Here's how the part is built. I have some questions about the finished solid (model axes, mm). A direction names the side the tool comes from. Coordinates: 2 decimals unless noted, no trailing zeros. Loops run counter-clockwise (first coordinate to the right, second up) from the corner with the lowest first, then second, coordinate; pieces in that order, holes last. Notation, with made-up numbers: M -9,-22 L -1,-22 A12 cw -1,-4 Z; hole C 38,-26 d1. An arc over 180 degrees is marked long. Use one line per item in the form item = value. Start each with the question number.
(1) Imagine slicing it at A-A, the plane x = 0. Please give me the cut outline in (y, z).
(2) Please list where these lines run through material, in increasing order: L1, parallel to Y at x = -15, z = 2.35; L2, parallel to Z at x = 1, y = -0.75; L3, parallel to X at y = 14.25, z = 1.5.
(3) On a 3-axis mill with a long thin cutter (end or side, diameter ignored), from which of +Z, -Z, +X, -X, +Y, -Y can I reach the whole of each face in a straight line? I mean faces 5 (the flat face through (19, 0, 6)), 6 (the flat face through (-19, 0, 6)), 7 (the cylindrical face through (10.5, 0, 11.9)), 8 (the flat face through (0, 0, 18)). Say none if no direction works.
(4) Imagine slicing it at B-B, the plane z = 2.25. Please give me the cut outline in (x, y), and give its area (3 significant figures).
(5) Imagine slicing it at D-D, the plane y = 2. Please give me the cut outline in (x, z).
(6) Imagine slicing it at C-C, the plane y = 5.75. Please give me the cut outline in (x, z), and give its area (3 significant figures).
(7) Thinking about a two-plate mould opening in Z: for faces 1 (the flat face through (0, 0, 15)), 2 (the flat face through (-13.5, 0, 11.5)), 3 (the cylindrical face through (15, 0.04, 7.43)), 4 (the flat face through (0, 0, 9)), which applies, +Z half, -Z half, draft (parallel to the pull), parting line (faces both ways), or undercut?
(8) Will these pins go through, and if not, where does the flat tip stop? P1, Ø2, axis at y = 17, z = 2.5, coming from the -X side; P2, Ø5, axis at x = -12.5, y = 16, coming from the +Z side; P3, Ø0.8, axis at y = -1, z = 11.5, coming from the -X side.
```python
from build123d import *

# Parameters (mm, degrees)
BASE_PLATE_DEPTH        = 3
CLEVIS_LUGS_PROFILE_W   = 40
CLEVIS_LUGS_PROFILE_H   = 6
CLEVIS_LUGS_PROFILE_R   = 5
CLEVIS_LUGS_PROFILE_R_2 = 2.5
CLEVIS_LUGS_DEPTH       = 3


with BuildPart() as part:
    # Base Plate Profile → Base Plate (new, symmetric)
    with BuildSketch(Plane(origin=(0, 0, 0), x_dir=(1, 0, 0), z_dir=(0, 1, 0))):
        with BuildLine():
            Line((-20, 0), (20, 0))
            Line((20, 0), (20, -6))
            Line((20, -6), (18.5, -6))
            ThreePointArc((18.5, -6), (14.964466094, -7.464466094), (13.5, -11))
            Line((13.5, -11), (13.5, -12))
            ThreePointArc((13.5, -12), (11.742640687, -16.242640687), (7.5, -18))
            Line((7.5, -18), (-7.5, -18))
            ThreePointArc((-7.5, -18), (-11.742640687, -16.242640687), (-13.5, -12))
            Line((-13.5, -12), (-13.5, -11))
            ThreePointArc((-13.5, -11), (-14.964466094, -7.464466094), (-18.5, -6))
            Line((-18.5, -6), (-20, -6))
            Line((-20, -6), (-20, 0))
        make_face()
        with BuildLine():
            Line((-7.5, -9), (7.5, -9))
            ThreePointArc((7.5, -9), (10.5, -12), (7.5, -15))
            Line((7.5, -15), (-7.5, -15))
            ThreePointArc((-7.5, -15), (-10.5, -12), (-7.5, -9))
        make_face(mode=Mode.SUBTRACT)
    extrude(amount=BASE_PLATE_DEPTH, both=True)

    # Clevis Lugs Profile → Clevis Lugs (add, symmetric)
    # profile 1 of 5: a face of its own
    with BuildSketch(Plane(origin=(0, 0, 0), x_dir=(-1, 0, 0), z_dir=(0, 0, -1))):
        Rectangle(CLEVIS_LUGS_PROFILE_W, CLEVIS_LUGS_PROFILE_H)
    # profile 2 of 5: a face of its own
    with BuildSketch(Plane(origin=(0, 0, 0), x_dir=(-1, 0, 0), z_dir=(0, 0, -1))):
        with BuildLine():
            Line((-20, 15), (-20, 3))
            Line((-20, 3), (-5, 3))
            ThreePointArc((-5, 3), (-8.535533906, 4.464466094), (-10, 8))
            Line((-10, 8), (-10, 15))
            ThreePointArc((-10, 15), (-15, 10), (-20, 15))
        make_face()
    # profile 3 of 5: a face of its own
    with BuildSketch(Plane(origin=(0, 0, 0), x_dir=(-1, 0, 0), z_dir=(0, 0, -1))):
        with BuildLine():
            Line((5, 3), (20, 3))
            Line((20, 3), (20, 15))
            ThreePointArc((20, 15), (15, 10), (10, 15))
            Line((10, 15), (10, 8))
            ThreePointArc((10, 8), (8.535533906, 4.464466094), (5, 3))
        make_face()
    # profile 4 of 5: a face of its own
    with BuildSketch(Plane(origin=(0, 0, 0), x_dir=(-1, 0, 0), z_dir=(0, 0, -1))):
        with Locations((15, 15)):
            Circle(CLEVIS_LUGS_PROFILE_R)
        with Locations((15, 15)):
            Circle(CLEVIS_LUGS_PROFILE_R_2, mode=Mode.SUBTRACT)
    # profile 5 of 5: a face of its own
    with BuildSketch(Plane(origin=(0, 0, 0), x_dir=(-1, 0, 0), z_dir=(0, 0, -1))):
        with Locations((-15, 15)):
            Circle(CLEVIS_LUGS_PROFILE_R)
        with Locations((-15, 15)):
            Circle(CLEVIS_LUGS_PROFILE_R_2, mode=Mode.SUBTRACT)
    extrude(amount=CLEVIS_LUGS_DEPTH, both=True)


solid = part.part
```
Answer:
q1.outline = M -3,-3 L 3,-3 L 3,9 L -3,9 Z; M -3,15 L 3,15 L 3,18 L -3,18 Z
q2.L1 = -3 to 12.5, 17.5 to 20
q2.L2 = -3 to 9, 15 to 18
q2.L3 = -20 to -17.38, -12.62 to -10, 10 to 12.62, 17.38 to 20
q3.face_5 = +Z, +X, +Y, -Y
q3.face_6 = +Z, -X, +Y, -Y
q3.face_7 = +Y, -Y
q3.face_8 = +Z, +X, -X, +Y, -Y
q4.outline = M -20,-3 L 20,-3 L 20,15 A5 ccw 10,15 L 10,8 A5 cw 5,3 L -5,3 A5 cw -10,8 L -10,15 A5 ccw -20,15 Z; hole C -15,15 d5; hole C 15,15 d5
q4.area = 530 mm²
q5.outline = M -20,-3 L 20,-3 L 20,6 L 18.5,6 A5 cw 13.5,11 L 13.5,12 A6 ccw 7.5,18 L -7.5,18 A6 ccw -13.5,12 L -13.5,11 A5 cw -18.5,6 L -20,6 Z; hole M -7.5,9 L 7.5,9 A3 ccw 7.5,15 L -7.5,15 A3 ccw Z
q6.outline = M -20,-3 L -9.47,-3 L -9.47,3 L -20,3 Z; M 9.47,-3 L 20,-3 L 20,3 L 9.47,3 Z
q6.area = 126 mm²
q7.face_1 = undercut
q7.face_2 = draft
q7.face_3 = +Z half
q7.face_4 = undercut
q8.P1 = -19.9
q8.P2 = 3
q8.P3 = -13.5
